Read the model definition and answer for the solid it produces. Units are mm, in the model's axes. Face numbers are marked on the shaded views. A direction names the side the tool comes from. Coordinates: 2 decimals unless noted, no trailing zeros. Order: outer loops, then holes, each group sorted by start corner. A loop starts at its lowest first (then second) coordinate and runs counter-clockwise, first axis right, second up. Notation, with made-up numbers: (-1.5, 37) -> (43.5, 37) arc R19 cw to (43.5, 61) -> close; hole circle Ø8 at (47, -36.75). An arc over 180 degrees is marked (long way). Use CSV: the item, a comma, the result in double quotes.
```python
from build123d import *

# Parameters (mm, degrees)
SKETCH_1_W          = 80
SKETCH_1_H          = 80
EXTRUDE_1_DEPTH     = 50
SKETCH_2_R          = 35
CUT_EXTRUDE_1_DEPTH = 1
FILLET_1_R          = 2
HOLE_WIZARD_M5_1_D  = 4.2
SKETCH_10_R         = 5
CUT_EXTRUDE_2_DEPTH = 20
SKETCH_11_R         = 5
EXTRUDE_3_DEPTH     = 32
SKETCH_13_W         = 4
SKETCH_13_H         = 5
CUT_EXTRUDE_4_DEPTH = 25
SKETCH_14_R         = 15
EXTRUDE_4_DEPTH     = 1


with BuildPart() as part:
    # Sketch 1 → Extrude 1 (new body)
    with BuildSketch(Plane.XY):
        with Locations((40, 40)):
            Rectangle(SKETCH_1_W, SKETCH_1_H)
    extrude(amount=EXTRUDE_1_DEPTH)

    # Sketch 2 → Cut-Extrude 1 (cut)
    with BuildSketch(Plane.XY.offset(50)):
        with Locations((40, 40)):
            Circle(SKETCH_2_R)
    extrude(amount=-CUT_EXTRUDE_1_DEPTH, mode=Mode.SUBTRACT)

    # Fillet 1
    fillet_1_edges = [part.edges().sort_by_distance(p)[0] for p in [
        (0, 80, 25),
        (80, 80, 25),
        (80, 0, 25),
        (0, 0, 25),
    ]]
    fillet(fillet_1_edges, radius=FILLET_1_R)

    # Hole Wizard M5 _1 (through all)
    with Locations(Plane(origin=(73.234018716, 73.234018716, 0), x_dir=(-1, 0, 0), z_dir=(0, 0, -1))):
        with Locations((0, 0), (66.468037432, 0), (66.468037432, -66.468037432), (0, -66.468037432)):
            Hole(HOLE_WIZARD_M5_1_D / 2)

    # Sketch 10 → Cut-Extrude 2 (cut)
    with BuildSketch(Plane(origin=(0, 0, 0), x_dir=(-1, 0, 0), z_dir=(0, 0, -1))):
        with Locations((-40, 40)):
            Circle(SKETCH_10_R)
    extrude(amount=-CUT_EXTRUDE_2_DEPTH, mode=Mode.SUBTRACT)



with BuildPart() as body_2:
    # Sketch 11 → Extrude 3 (new body)
    with BuildSketch(Plane.XY.offset(50)):
        with Locations((40, 25)):
            Circle(SKETCH_11_R)
    extrude(amount=EXTRUDE_3_DEPTH)

    # Sketch 13 → Cut-Extrude 4 (cut)
    with BuildSketch(Plane.XY.offset(82)):
        with Locations((40, 20)):
            Rectangle(SKETCH_13_W, SKETCH_13_H)
    extrude(amount=-CUT_EXTRUDE_4_DEPTH, mode=Mode.SUBTRACT)


with BuildPart() as part_1:
    add(part.part)

    add(body_2.part)  # Extrude 4 merges body 2
    # Sketch 14 → Extrude 4 (add)
    with BuildSketch(Plane.XY.offset(49)):
        with Locations((40, 25)):
            Circle(SKETCH_14_R)
    extrude(amount=EXTRUDE_4_DEPTH)


solid = part_1.part
```
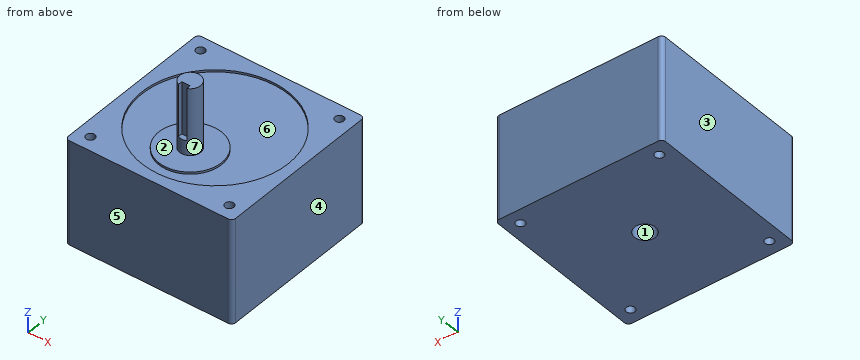
Item 1: Find section C-C, the plane z = 10.5. Give the vertices of the cut face in (x, y).
Return value:
outline,"(0, 2) arc R2 ccw to (2, 0) -> (78, 0) arc R2 ccw to (80, 2) -> (80, 78) arc R2 ccw to (78, 80) -> (2, 80) arc R2 ccw to (0, 78) -> close; hole circle Ø4.2 at (6.77, 6.77); hole circle Ø4.2 at (6.77, 73.23); hole circle Ø10 at (40, 40); hole circle Ø4.2 at (73.23, 6.77); hole circle Ø4.2 at (73.23, 73.23)"
Item 2: A tool of negligible diameter and unlimited length cuts with its end or side. For the marked faces 1, 2 and 3, from which of +Z, -Z, +X, -X, +Y, -Y can it reach the whole face along a straight path? Write none if from no direction.
Return value:
face 1,"-Z"
face 2,"+Z"
face 3,"+Z, -Z, -X, +Y, -Y"
Item 3: Find section D-D, the plane y = 66.5. Give the vertices of the cut face in (x, z).
Return value:
outline,"(0, 0) -> (80, 0) -> (80, 50) -> (62.86, 50) -> (62.86, 49) -> (17.14, 49) -> (17.14, 50) -> (0, 50) -> close"
Item 4: Straight lines are drawn through the part: line 1 along Y through (x, z) = (40, 14.25); line 2 along Z through (x, y) = (74.5, 19); line 3 along Z through (x, y) = (26, 34). For each, find the intervals that lie inside material, in ascending order.
Return value:
line 1,"y = 0 to 35, 45 to 80"
line 2,"z = 0 to 50"
line 3,"z = 0 to 49"
Item 5: Each of these flat-tipped pins is pushed along its axis until it touches: P1, Ø21, axis at x = 46, y = 45.5, coming from the +Z side; P2, Ø4.5, axis at x = 40.5, z = 71.5, coming from the -Y side; P3, Ø4, axis at x = 22.5, y = 35.5, coming from the +Z side. Where does it stop, or does it pass through?
Return value:
P1,"stops at z = 50"
P2,"stops at y = 20.42"
P3,"stops at z = 49"
Item 6: Find section B-B, the plane y = 25. Give the vertices of the cut face in (x, z), then the cut area to 3 significant figures.
Return value:
outline,"(0, 0) -> (80, 0) -> (80, 50) -> (71.62, 50) -> (71.62, 49) -> (55, 49) -> (55, 50) -> (45, 50) -> (45, 82) -> (35, 82) -> (35, 50) -> (25, 50) -> (25, 49) -> (8.38, 49) -> (8.38, 50) -> (0, 50) -> close"
area,"4,290 mm^2"
Item 7: Find section A-A, the plane x = 40. Give the vertices of the cut face in (y, z), then the cut area to 3 significant figures.
Return value:
outline,"(0, 0) -> (35, 0) -> (35, 20) -> (45, 20) -> (45, 0) -> (80, 0) -> (80, 50) -> (75, 50) -> (75, 49) -> (40, 49) -> (40, 50) -> (30, 50) -> (30, 82) -> (22.5, 82) -> (22.5, 57) -> (20, 57) -> (20, 50) -> (10, 50) -> (10, 49) -> (5, 49) -> (5, 50) -> (0, 50) -> close"
area,"4,020 mm^2"
Item 8: The mould has two halves that part along Y. Classify the marked faces 4, 5, 6 and 7: +Y half, -Y half, draft (parallel to the pull), parting line (faces both ways), or undercut.
Return value:
face 4,"draft"
face 5,"-Y half"
face 6,"undercut"
face 7,"parting line"
